Input: part model. Units: mm. Frame: model coordinates. A direction names the side the tool comes from. Coordinates: 2 decimals unless noted, no trailing zeros. Order: outer loops, then holes, each group sorted by start corner. A loop starts at its lowest first (then second) coordinate and runs counter-clockwise, first axis right, second up. Notation, with made-up numbers: (73.25, 39) -> (107.25, 39) arc R23 cw to (107.25, 64) -> close; hole circle Ø3 at (-33, 50.25). An arc over 180 degrees is marked (long way). Write each question's results on one line, items separated by ' | '.
```python
from build123d import *

# Parameters (mm, degrees)
SKETCH_1_W                     = 108
SKETCH_1_H                     = 675
EXTRUDE_1_DEPTH                = 10
HOLE_WIZARD_M6_1_D             = 5
HOLE_WIZARD_M6_1_2_D           = 6.6
HOLE_WIZARD_M6_1_2_CBORE_D     = 11
HOLE_WIZARD_M6_1_2_CBORE_DEPTH = 6.4
HOLE_WIZARD_M5_1_D             = 4.2
HOLE_WIZARD_M5_1_DEPTH         = 14
HOLE_WIZARD_M5_1_TIP           = 1.2618073
HOLE_WIZARD_M6_2_D             = 5
HOLE_WIZARD_M6_2_DEPTH         = 17
HOLE_WIZARD_M6_2_TIP           = 1.502151548
HOLE_WIZARD_M5_1_2_D           = 5.5
HOLE_WIZARD_M5_1_2_DEPTH       = 14
HOLE_WIZARD_M5_1_2_CBORE_D     = 10
HOLE_WIZARD_M5_1_2_CBORE_DEPTH = 5.4
HOLE_WIZARD_M5_1_2_TIP         = 1.652366702
HOLE_WIZARD_M6_3_D             = 5
HOLE_WIZARD_M6_3_DEPTH         = 17
HOLE_WIZARD_M6_3_TIP           = 1.502151548
SKETCH_14_R                    = 5.5
CUT_EXTRUDE_1_DEPTH            = 60
SKETCH_15_R                    = 2.5
SKETCH_15_W                    = 30
SKETCH_15_H                    = 90
SKETCH_15_R_2                  = 5
CUT_EXTRUDE_2_DEPTH            = 684.658540501
CHAMFER_1_SIZE                 = 5
HOLE_WIZARD_M6_4_D             = 5


with BuildPart() as part:
    # 草图1 → 凸台-拉伸1 (new body)
    with BuildSketch(Plane.XY):
        with Locations((54, 337.5)):
            Rectangle(SKETCH_1_W, SKETCH_1_H)
    extrude(amount=EXTRUDE_1_DEPTH)

    # Hole Wizard M6 _1 (through all)
    with Locations(Plane.XY.offset(10)):
        with Locations((10, 645), (10, 625), (10, 50), (10, 30)):
            Hole(HOLE_WIZARD_M6_1_D / 2)

    # Hole Wizard M6 _1 2 (through all)
    with Locations(Plane(origin=(0, 0, 0), x_dir=(-1, 0, 0), z_dir=(0, 0, -1))):
        with Locations((-45, 513.5), (-5, 513.5), (-45, 473.5), (-5, 473.5), (-5, 201.5), (-45, 201.5), (-5, 161.5), (-45, 161.5)):
            CounterBoreHole(HOLE_WIZARD_M6_1_2_D / 2, HOLE_WIZARD_M6_1_2_CBORE_D / 2, HOLE_WIZARD_M6_1_2_CBORE_DEPTH)

    # Hole Wizard M5 _1
    with Locations(Plane.XY.offset(10)):
        with Locations((29.5, 354.5), (73.5, 354.5), (29.5, 320.5), (73.5, 320.5)):
            Hole(HOLE_WIZARD_M5_1_D / 2, depth=HOLE_WIZARD_M5_1_DEPTH)
            with Locations((0, 0, -(HOLE_WIZARD_M5_1_DEPTH + HOLE_WIZARD_M5_1_TIP / 2))):  # 118° drill point
                Cone(0, HOLE_WIZARD_M5_1_D / 2, HOLE_WIZARD_M5_1_TIP, mode=Mode.SUBTRACT)

    # M6 螺纹孔2
    with Locations(Plane.XY.offset(10)):
        with Locations((97.5, 431.5), (97.5, 396.5)):
            Hole(HOLE_WIZARD_M6_2_D / 2, depth=HOLE_WIZARD_M6_2_DEPTH)
            with Locations((0, 0, -(HOLE_WIZARD_M6_2_DEPTH + HOLE_WIZARD_M6_2_TIP / 2))):  # 118° drill point
                Cone(0, HOLE_WIZARD_M6_2_D / 2, HOLE_WIZARD_M6_2_TIP, mode=Mode.SUBTRACT)

    # Hole Wizard M5 _1 2
    with Locations(Plane.XY.offset(10)):
        with Locations((61.5, 367.5), (91.5, 367.5), (61.5, 307.5), (91.5, 307.5)):
            CounterBoreHole(HOLE_WIZARD_M5_1_2_D / 2, HOLE_WIZARD_M5_1_2_CBORE_D / 2, HOLE_WIZARD_M5_1_2_CBORE_DEPTH, depth=HOLE_WIZARD_M5_1_2_DEPTH)
            with Locations((0, 0, -(HOLE_WIZARD_M5_1_2_DEPTH + HOLE_WIZARD_M5_1_2_TIP / 2))):  # 118° drill point
                Cone(0, HOLE_WIZARD_M5_1_2_D / 2, HOLE_WIZARD_M5_1_2_TIP, mode=Mode.SUBTRACT)

    # M6 螺纹孔3
    with Locations(Plane(origin=(0, 0, 0), x_dir=(-1, 0, 0), z_dir=(0, 0, -1))):
        with Locations((-38, 380), (-10, 380), (-38, 295), (-10, 295)):
            Hole(HOLE_WIZARD_M6_3_D / 2, depth=HOLE_WIZARD_M6_3_DEPTH)
            with Locations((0, 0, -(HOLE_WIZARD_M6_3_DEPTH + HOLE_WIZARD_M6_3_TIP / 2))):  # 118° drill point
                Cone(0, HOLE_WIZARD_M6_3_D / 2, HOLE_WIZARD_M6_3_TIP, mode=Mode.SUBTRACT)

    # 草图14 → 切除-拉伸1 (cut)
    with BuildSketch(Plane.XY.offset(10)):
        with Locations((41.5, 444)):
            Circle(SKETCH_14_R)
        with Locations((6.5, 444)):
            Circle(SKETCH_14_R)
        with Locations((41.5, 409)):
            Circle(SKETCH_14_R)
        with Locations((6.5, 409)):
            Circle(SKETCH_14_R)
        with Locations((41.5, 266)):
            Circle(SKETCH_14_R)
        with Locations((41.5, 231)):
            Circle(SKETCH_14_R)
        with Locations((6.5, 231)):
            Circle(SKETCH_14_R)
        with Locations((6.5, 266)):
            Circle(SKETCH_14_R)
    extrude(amount=-CUT_EXTRUDE_1_DEPTH, mode=Mode.SUBTRACT)

    # 草图15 → 切除-拉伸2 (cut, through all)
    # profile 1 of 5: a face of its own
    with BuildSketch(Plane.XY.offset(10)):
        Polygon((108, 382.5), (108, 675), (58, 675), (58, 382.5), (78, 382.5), align=None)
        with Locations((97.5, 396.5)):
            Circle(SKETCH_15_R, mode=Mode.SUBTRACT)
        with Locations((97.5, 431.5)):
            Circle(SKETCH_15_R, mode=Mode.SUBTRACT)
    # profile 2 of 5: a face of its own
    with BuildSketch(Plane.XY.offset(10)):
        with Locations((93, 337.5)):
            Rectangle(SKETCH_15_W, SKETCH_15_H)
        with Locations((91.5, 307.5)):
            Circle(SKETCH_15_R_2, mode=Mode.SUBTRACT)
        with Locations((91.5, 367.5)):
            Circle(SKETCH_15_R_2, mode=Mode.SUBTRACT)
    # profile 3 of 5: a face of its own
    with BuildSketch(Plane.XY.offset(10)):
        Polygon((108, 0), (108, 292.5), (78, 292.5), (58, 292.5), (58, 0), align=None)
    # profile 4 of 5: a face of its own
    with BuildSketch(Plane.XY.offset(10)):
        with Locations((91.5, 367.5)):
            Circle(SKETCH_15_R_2)
    # profile 5 of 5: a face of its own
    with BuildSketch(Plane.XY.offset(10)):
        with Locations((91.5, 307.5)):
            Circle(SKETCH_15_R_2)
    extrude(amount=-CUT_EXTRUDE_2_DEPTH, mode=Mode.SUBTRACT)

    # 倒角1
    chamfer_1_edges = [part.edges().sort_by_distance(p)[0] for p in [
        (58, 675, 5),
        (58, 0, 5),
        (78, 292.5, 5),
        (78, 382.5, 5),
    ]]
    chamfer(chamfer_1_edges, length=CHAMFER_1_SIZE)

    # M6 螺纹孔4 (through all)
    with Locations(Plane.XY.offset(10)):
        with Locations((15.5, 142), (15.5, 107)):
            Hole(HOLE_WIZARD_M6_4_D / 2)


solid = part.part
```
(1) Pin query (flat end, axial travel): P1, Ø3, axis at y = 388, z = 6.5, coming from the +X side; P2, Ø8, axis at x = 61.5, y = 367.5, coming from the +Z side. Return the tip coordinate at first contact, or that it passes through.
Return value:
P1: x = 58 | P2: z = 4.6
(2) Cut plane A-A, the plane y = 266. Return loops of the section in (x, z).
Return value:
outline: (0, 0) -> (1, 0) -> (1, 10) -> (0, 10) -> close; (12, 0) -> (36, 0) -> (36, 10) -> (12, 10) -> close; (47, 0) -> (58, 0) -> (58, 10) -> (47, 10) -> close
(3) Line query: line 1 along X through (y, z) = (444, 6.75); line 2 along X through (y, z) = (473.5, 8.2); line 3 along Y through (x, z) = (41, 6.75). Output: solid intervals per line, ascending. Write a range as from..to.
Return value:
line 1: 0..1, 12..36, 47..58 | line 2: 0..1.7, 8.3..41.7, 48.3..58 | line 3: 0..225.52, 236.48..260.52, 271.48..403.52, 414.48..438.52, 449.48..675
(4) Mould query, pull axis Y, two halves, no side actions, for faces 3 (the face through (5.31, 403.63, 5.07)), 4 (the face through (30, 342, 10)). Classes: +Y half, -Y half, draft (parallel to the pull), parting line (faces both ways), or undercut.
Return value:
face 3: undercut | face 4: draft
(5) Cut plane B-B, the plane y = 582. Return loops of the section in (x, z), plus the area to 3 significant figures.
Return value:
outline: (0, 0) -> (58, 0) -> (58, 10) -> (0, 10) -> close | area: 580 mm2
(6) Reachability of faces 1 (the face through (10.496, 473.709, 3.155)), 2 (the face through (40.31, 260.63, 5.07)) from +Z, -Z, +X, -X, +Y, -Y: full face, straight path, thin tool, end or side. Return the list, or none.
Return value:
face 1: -Z | face 2: +Z, -Z
